The listing builds one solid part. Answer for the finished solid, in the listing's coordinates (mm). A direction names the side the tool comes from. Round coordinates to 2 decimals unless told otherwise and drop trailing zeros. Order: outer loops, then holes, each group sorted by start corner. A loop starts at its lowest first (then second) coordinate and runs counter-clockwise, first axis right, second up. Notation, with made-up numbers: (82, 6) - (91, 6) arc R9 ccw to (91, 16) - close; hole circle Ø5 at (-38, 41). An arc over 180 degrees is marked (long way). One line per item, written item: value. Start each with the question number.
1. Section D-D, the plane x = 134.5 is taken. Give the vertices of the cut face in (y, z), then the cut area to 3 significant figures.
2. A tool of negligible diameter and unlimited length cuts with its end or side. For faces 4 (the flat face through (-150, 0, -31)), 5 (the cylindrical face through (-28.828, -4.577, 21.077)), 6 (the cylindrical face through (-125, 0, 15)), from which of +Z, -Z, +X, -X, +Y, -Y can it reach the whole face along a straight path? Write none if from no direction.
3. Straight lines are drawn through the part: line 1 (X direction, y = 3, z = 30); line 2 (Z direction, x = -30, y = -4); line 3 (Y direction, x = 145, z = -11.75). For each, find the intervals that lie inside material, in ascending order.
4. For a pull along X with two mould halves and no side action, classify faces 1 (the flat face through (149, 0, 1.25)), 2 (the flat face through (155, 0, 19)), 3 (the flat face through (140, 0, -31)) as released by +X, released by -X, zero draft, split by the parting line, or undercut.
5. Flat-ended cylindrical pins translate along their axes: P1, Ø14.5, axis at x = -27.5, z = -26, coming from the -Y side; P2, Ø10.5, axis at x = 145, y = 0, coming from the -Z side. Find the tip coordinate at first contact, or state that the pin passes through.
6. Section A-A, the plane z = 30 is taken. Give the vertices of the cut face in (x, y).
7. Section B-B, the plane x = 30 is taken. Give the vertices of the cut face in (y, z).
8. Section C-C, the plane x = -80 is taken. Give the vertices of the cut face in (y, z), then the cut area to 3 significant figures.
from build123d import *

# Parameters (mm, degrees)
SKETCH_1_W                  = 310
SKETCH_1_H                  = 80
EXTRUDE_1_DEPTH             = 10
SKETCH_2_R                  = 15
CUT_EXTRUDE_1_DEPTH         = 20
CHAMFER_1_SIZE              = 3
CUT_EXTRUDE_2_DEPTH         = 20
HOLE_WIZARD_2_D             = 9
HOLE_WIZARD_2_DEPTH         = 40
HOLE_WIZARD_2_CBORE_D       = 15
HOLE_WIZARD_2_CBORE_DEPTH   = 9
HOLE_WIZARD_2_TIP           = 2.703872786
HOLE_WIZARD_M8_1_D          = 6.8
HOLE_WIZARD_M8_1_DEPTH      = 19.75
HOLE_WIZARD_M8_1_TIP        = 2.042926105
HOLE_WIZARD_2_2_D           = 11
HOLE_WIZARD_2_2_DEPTH       = 19.75
HOLE_WIZARD_2_2_CBORE_D     = 18
HOLE_WIZARD_2_2_CBORE_DEPTH = 11
HOLE_WIZARD_2_2_TIP         = 3.304733405
HOLE_WIZARD_M12_1_D         = 10.2


with BuildPart() as part:
    # 草图1 → 凸台-拉伸1 (new, symmetric)
    with BuildSketch(Plane(origin=(0, 0, 0), x_dir=(1, 0, 0), z_dir=(0, 1, 0))):
        Rectangle(SKETCH_1_W, SKETCH_1_H)
    extrude(amount=EXTRUDE_1_DEPTH, both=True)

    # 草图2 → 切除-拉伸1 (cut)
    with BuildSketch(Plane(origin=(0, 10, 0), x_dir=(1, 0, 0), z_dir=(0, 1, 0))):
        with Locations(Location((125, 0, 0), (0, 0, 270))):
            Circle(SKETCH_2_R)
        with Locations(Location((-125, 0, 0), (0, 0, 90))):
            Circle(SKETCH_2_R)
    extrude(amount=-CUT_EXTRUDE_1_DEPTH, mode=Mode.SUBTRACT)

    # 倒角1
    chamfer_1_edges = [part.edges().sort_by_distance(p)[0] for p in [
        (155, 0, 40),
        (-155, 0, 40),
        (-155, 0, -40),
        (155, 0, -40),
    ]]
    chamfer(chamfer_1_edges, length=CHAMFER_1_SIZE)

    # 草图3 → 切除-拉伸2 (cut)
    with BuildSketch(Plane(origin=(0, 10, 0), x_dir=(1, 0, 0), z_dir=(0, 1, 0))):
        with BuildLine():
            Line((155, -1.25), (103, -1.25))
            ThreePointArc((103, -1.25), (101.75, 0), (103, 1.25))
            Line((103, 1.25), (155, 1.25))
            ThreePointArc((155, 1.25), (156.25, 0), (155, -1.25))
        make_face()
        with BuildLine():
            Line((-155, -1.25), (-103, -1.25))
            ThreePointArc((-103, -1.25), (-101.75, 0), (-103, 1.25))
            Line((-103, 1.25), (-155, 1.25))
            ThreePointArc((-155, 1.25), (-156.25, 0), (-155, -1.25))
        make_face()
    extrude(amount=-CUT_EXTRUDE_2_DEPTH, mode=Mode.SUBTRACT)

    # Hole Wizard 2
    with Locations(Plane(origin=(0, 0, -40), x_dir=(-1, 0, 0), z_dir=(0, 0, -1))):
        with Locations((-145, 0), (145, 0)):
            CounterBoreHole(HOLE_WIZARD_2_D / 2, HOLE_WIZARD_2_CBORE_D / 2, HOLE_WIZARD_2_CBORE_DEPTH, depth=HOLE_WIZARD_2_DEPTH)
            with Locations((0, 0, -(HOLE_WIZARD_2_DEPTH + HOLE_WIZARD_2_TIP / 2))):  # 118° drill point
                Cone(0, HOLE_WIZARD_2_D / 2, HOLE_WIZARD_2_TIP, mode=Mode.SUBTRACT)

    # M8 螺纹孔1
    with Locations(Plane(origin=(0, 0, 1.25), x_dir=(-1, 0, 0), z_dir=(0, 0, -1))):
        with Locations((-145, 0), (145, 0)):
            Hole(HOLE_WIZARD_M8_1_D / 2, depth=HOLE_WIZARD_M8_1_DEPTH)
            with Locations((0, 0, -(HOLE_WIZARD_M8_1_DEPTH + HOLE_WIZARD_M8_1_TIP / 2))):  # 118° drill point
                Cone(0, HOLE_WIZARD_M8_1_D / 2, HOLE_WIZARD_M8_1_TIP, mode=Mode.SUBTRACT)

    # Hole Wizard 2 2
    with Locations(Plane(origin=(0, -10, 0), x_dir=(-1, 0, 0), z_dir=(0, -1, 0))):
        with Locations((-30, 30), (30, 30), (30, -30), (-30, -30)):
            CounterBoreHole(HOLE_WIZARD_2_2_D / 2, HOLE_WIZARD_2_2_CBORE_D / 2, HOLE_WIZARD_2_2_CBORE_DEPTH, depth=HOLE_WIZARD_2_2_DEPTH)
            with Locations((0, 0, -(HOLE_WIZARD_2_2_DEPTH + HOLE_WIZARD_2_2_TIP / 2))):  # 118° drill point
                Cone(0, HOLE_WIZARD_2_2_D / 2, HOLE_WIZARD_2_2_TIP, mode=Mode.SUBTRACT)

    # M12 螺纹孔1 (through all)
    with Locations(Plane(origin=(0, 10, 0), x_dir=(1, 0, 0), z_dir=(0, 1, 0))):
        with Locations((80, 0), (-80, 0)):
            Hole(HOLE_WIZARD_M12_1_D / 2)


solid = part.part
Answer list:
1. outline: (-10, -40) - (10, -40) - (10, -11.61) - (-10, -11.61) - close; (-10, 11.61) - (10, 11.61) - (10, 40) - (-10, 40) - close
1. area: 1,140 mm²
2. face 4: -Z
2. face 5: -Y
2. face 6: +Y, -Y
3. line 1: x = -155 to -35.5, -24.5 to 24.5, 35.5 to 155
3. line 2: z = -40 to -39, -21 to 21, 39 to 40
3. line 3: y = -10 to -4.5, 4.5 to 10
4. face 1: zero draft
4. face 2: released by +X
4. face 3: undercut
5. P1: stops at y = -10
5. P2: stops at z = -31
6. outline: (-155, -10) - (-39, -10) - (-39, 1) - (-35.5, 1) - (-35.5, 9.75) - (-35.08, 10) - (-155, 10) - close; (-24.92, 10) - (-24.5, 9.75) - (-24.5, 1) - (-21, 1) - (-21, -10) - (21, -10) - (21, 1) - (24.5, 1) - (24.5, 9.75) - (24.92, 10) - close; (35.08, 10) - (35.5, 9.75) - (35.5, 1) - (39, 1) - (39, -10) - (155, -10) - (155, 10) - close
7. outline: (-10, -40) - (10, -40) - (10, -35.08) - (9.75, -35.5) - (1, -35.5) - (1, -39) - (-10, -39) - close; (-10, -21) - (1, -21) - (1, -24.5) - (9.75, -24.5) - (10, -24.92) - (10, 24.92) - (9.75, 24.5) - (1, 24.5) - (1, 21) - (-10, 21) - close; (-10, 39) - (1, 39) - (1, 35.5) - (9.75, 35.5) - (10, 35.08) - (10, 40) - (-10, 40) - close
8. outline: (-10, -40) - (10, -40) - (10, -5.1) - (-10, -5.1) - close; (-10, 5.1) - (10, 5.1) - (10, 40) - (-10, 40) - close
8. area: 1,400 mm²
